```python
from build123d import *

# Parameters (mm, degrees)
BASE_PLATE_PROFILE_R                 = 7
BASE_PLATE_WITH_MOUNTING_HOLES_DEPTH = 15
BEARING_BOSS_PROFILE_R               = 20
BEARING_BOSS_DEPTH                   = 50
BORE_PROFILE_R                       = 10
BEARING_BORE_DEPTH                   = 243
SUPPORT_RIB_REACH                    = 102.125
SUPPORT_RIB_PROFILE_WALL_W           = 248.347566232
SUPPORT_RIB_PROFILE_WALL_H           = 10


with BuildPart() as part:
    # Base Plate Profile → Base Plate with Mounting Holes (new body)
    with BuildSketch(Plane(origin=(0, 0, 0), x_dir=(1, 0, 0), z_dir=(0, 1, 0))):
        with BuildLine():
            Line((70, 20), (70, -20))
            ThreePointArc((70, -20), (67.071067812, -27.071067812), (60, -30))
            Line((60, -30), (-60, -30))
            ThreePointArc((-60, -30), (-67.071067812, -27.071067812), (-70, -20))
            Line((-70, -20), (-70, 20))
            ThreePointArc((-70, 20), (-67.071067812, 27.071067812), (-60, 30))
            Line((-60, 30), (60, 30))
            ThreePointArc((60, 30), (67.071067812, 27.071067812), (70, 20))
        make_face()
        with Locations(Location((60, -20, 0), (0, 0, 270))):
            Circle(BASE_PLATE_PROFILE_R, mode=Mode.SUBTRACT)
        with Locations(Location((-60, 20, 0), (0, 0, 270))):
            Circle(BASE_PLATE_PROFILE_R, mode=Mode.SUBTRACT)
        with Locations(Location((60, 20, 0), (0, 0, 270))):
            Circle(BASE_PLATE_PROFILE_R, mode=Mode.SUBTRACT)
        with Locations(Location((-60, -20, 0), (0, 0, 270))):
            Circle(BASE_PLATE_PROFILE_R, mode=Mode.SUBTRACT)
    extrude(amount=BASE_PLATE_WITH_MOUNTING_HOLES_DEPTH)

    # Bearing Boss Profile → Bearing Boss (add)
    with BuildSketch(Plane(origin=(0, 15, 0), x_dir=(1, 0, 0), z_dir=(0, 1, 0))):
        with Locations(Location((0, 0, 0), (0, 0, 270))):
            Circle(BEARING_BOSS_PROFILE_R)
    extrude(amount=BEARING_BOSS_DEPTH)

    # Bore Profile → Bearing Bore (cut)
    with BuildSketch(Plane(origin=(0, 65, 0), x_dir=(1, 0, 0), z_dir=(0, 1, 0))):
        with Locations(Location((0, 0, 0), (0, 0, 270))):
            Circle(BORE_PROFILE_R)
    extrude(amount=-BEARING_BORE_DEPTH, mode=Mode.SUBTRACT)

    # Support Rib Profile wall → Support Rib (add, up to next)
    with BuildSketch(Plane(origin=(35, 32.5, 0), x_dir=(0.650791373456, -0.759256602365, 0), z_dir=(0.759256602365, 0.650791373456, 0)), mode=Mode.PRIVATE) as support_rib_sk1:
        Rectangle(SUPPORT_RIB_PROFILE_WALL_W, SUPPORT_RIB_PROFILE_WALL_H)
    support_rib_tool1 = extrude(support_rib_sk1.sketch, amount=-SUPPORT_RIB_REACH, mode=Mode.PRIVATE) - part.part
    support_rib = support_rib_tool1.solids().sort_by_distance((35, 32.5, 0))[0]
    add(support_rib)

    # Support Rib Mirror: Support Rib across plane
    add(support_rib.mirror(Plane(origin=(0, 0, 0), x_dir=(0, 0, 1), z_dir=(1, 0, 0))))


solid = part.part
```
Check sheet for the modelled part. Datum: model origin and axes. Units: mm. A direction names the side the tool comes from. Give positions to 0.01 mm unless a question says otherwise; leave off trailing zeros. Write each loop counter-clockwise with the first axis right and the second up, starting at its lowest first coordinate (ties: lowest second). Pieces come first, ordered by that corner, then holes. Notation, with made-up numbers: (14, 29.25) - (18, 29.25) arc R22 ccw to (18, 48.25) - close; hole circle Ø3 at (-29, -17). An arc over 180 degrees is marked (long way). Answer as a JSON object with one key per item and string values. Group by question number.
1) Release check for a two-part mould opening along X. For faces 6 (the face through (-53.06, 7.4, 19.09)), 7 (the face through (30, 29, 5)), 8 (the face through (67.15, 7.4, 26.99)) record: pulls with the +X half, pulls with the -X half, needs draft (parallel to the pull), parting line crosses it, or undercut.
2) Sectioned sample at B-B (y = 10.5). Record the cut outline in (x, z), then the cut area to 3 significant figures.
3) Sectioned sample at C-C (x = 0). Record the cut outline in (y, z), then the cut area to 3 significant figures.
4) Sectioned sample at D-D (z = -15.5). Record the cut outline in (x, y).
5) Thickness scan on probe 1 along X at (y, z) = (9.5, -20); probe 2 along X at (y, z) = (5.5, -14); probe 3 along Y at (x, z) = (38.5, -22). Record the ranges inside material, lowest first. Write a range as from..to.
6) Depth check by flat-ended pin: P1, Ø16, axis at x = -60, z = -20, coming from the +Y side; P2, Ø12, axis at y = 50, z = -18, coming from the +X side; P3, Ø3, axis at y = 34.5, z = -5, coming from the +X side. Enter the tip coordinate at first touch or a pass-through.
7) Access from +Z, -Z, +X, -X, +Y, -Y to the whole of each face (thin tool, end or side, straight path). Record for faces 1 (the face through (-30, 29, 5)), 2 (the face through (-30, 29, -5)), 3 (the face through (66.94, 7.4, 19.09)), 4 (the face through (30, 29, -5)), 5 (the face through (-7.66, 39.65, 18.475)).
8) Sectioned sample at A-A (z = 0). Record the cut outline in (x, y), then the cut area to 3 significant figures.
Geometry results:
{
 "1": {"face 6": "undercut", "face 7": "needs draft", "face 8": "pulls with the +X half"},
 "2": {"outline": "(-70, -20) arc R10 ccw to (-60, -30) - (60, -30) arc R10 ccw to (70, -20) - (70, 20) arc R10 ccw to (60, 30) - (-60, 30) arc R10 ccw to (-70, 20) - close; hole circle Ø14 at (-60, -20); hole circle Ø14 at (-60, 20); hole circle Ø20 at (0, 0); hole circle Ø14 at (60, -20); hole circle Ø14 at (60, 20)", "area": "7,380 mm^2"},
 "3": {"outline": "(0, -30) - (15, -30) - (15, -20) - (65, -20) - (65, -10) - (0, -10) - close; (0, 10) - (65, 10) - (65, 20) - (15, 20) - (15, 30) - (0, 30) - close", "area": "1,600 mm^2"},
 "4": {"outline": "(-70, 0) - (-65.36, 0) - (-65.36, 15) - (-70, 15) - close; (-54.64, 0) - (54.64, 0) - (54.64, 15) - (12.64, 15) - (12.64, 65) - (-12.64, 65) - (-12.64, 15) - (-54.64, 15) - close; (65.36, 0) - (70, 0) - (70, 15) - (65.36, 15) - close"},
 "5": {"probe 1": "x = -70..-67, -53..53, 67..70", "probe 2": "x = -70..-63.61, -56.39..56.39, 63.61..70", "probe 3": "y = 0..15"},
 "6": {"P1": "stops at y = 15", "P2": "stops at x = 16", "P3": "stops at x = 34.57"},
 "7": {"face 1": "+Z, -X, +Y", "face 2": "-Z, -X, +Y", "face 3": "+Y, -Y", "face 4": "-Z, +X, +Y", "face 5": "+Y"},
 "8": {"outline": "(-70, 0) - (-10, 0) - (-10, 65) - (-20, 65) - (-20, 50) - (-50, 15) - (-70, 15) - close; (10, 0) - (70, 0) - (70, 15) - (50, 15) - (20, 50) - (20, 65) - (10, 65) - close", "area": "3,850 mm^2"}
}
